Input: part model. Units: mm. Frame: model coordinates. A direction names the side the tool comes from. Give positions to 0.01 mm unless a question says otherwise; leave off trailing zeros. Loops run counter-clockwise (first coordinate to the right, second up) from the corner with the lowest first, then second, coordinate; pieces in that order, holes last.
from build123d import *

# Parameters (mm, degrees)
BASE_PLATE_DEPTH       = 1
UPRIGHT_PLATE_SKETCH_R = 1
UPRIGHT_PLATE_DEPTH    = 1
RIB_SKETCH_W           = 1
RIB_SKETCH_H           = 4
RIB_DEPTH              = 5
PIVOT_HUB_DEPTH        = 1
PIVOT_HUB_DEPTH_BACK   = 2
PIVOT_HUB_SKETCH_R     = 1.5
HUB_BORE_SKETCH_R      = 0.75
HUB_BORE_DEPTH         = 3
SLOT_CUT_DEPTH         = 3


with BuildPart() as part:
    # Base Plate Sketch → Base Plate (new body)
    with BuildSketch(Plane(origin=(0, 0, 0), x_dir=(1, 0, 0), z_dir=(0, 1, 0))):
        with BuildLine():
            Line((-4, 1.5), (-2.8, 1.5))
            ThreePointArc((-2.8, 1.5), (-2.234314575, 1.265685425), (-2, 0.7))
            Line((-2, 0.7), (-2, 0.3))
            ThreePointArc((-2, 0.3), (-2.234314575, -0.265685425), (-2.8, -0.5))
            Line((-2.8, -0.5), (-4, -0.5))
            Line((-4, -0.5), (-4, -3))
            Line((-4, -3), (4, -3))
            Line((4, -3), (4, -0.5))
            Line((4, -0.5), (2.8, -0.5))
            ThreePointArc((2.8, -0.5), (2.234314575, -0.265685425), (2, 0.3))
            Line((2, 0.3), (2, 0.7))
            ThreePointArc((2, 0.7), (2.234314575, 1.265685425), (2.8, 1.5))
            Line((2.8, 1.5), (4, 1.5))
            ThreePointArc((4, 1.5), (3.560660172, 2.560660172), (2.5, 3))
            Line((2.5, 3), (-2.5, 3))
            ThreePointArc((-2.5, 3), (-3.560660172, 2.560660172), (-4, 1.5))
        make_face()
    extrude(amount=BASE_PLATE_DEPTH)

    # Upright Plate Sketch → Upright Plate (add)
    with BuildSketch(Plane.XY.offset(3)):
        with BuildLine():
            Line((-4, 0), (4, 0))
            Line((4, 0), (4, 3))
            ThreePointArc((4, 3), (3.414213562, 4.414213562), (2, 5))
            Line((2, 5), (-2, 5))
            ThreePointArc((-2, 5), (-3.414213562, 4.414213562), (-4, 3))
            Line((-4, 3), (-4, 0))
        make_face()
        with Locations((-2, 3)):
            Circle(UPRIGHT_PLATE_SKETCH_R, mode=Mode.SUBTRACT)
        with Locations((2, 3)):
            Circle(UPRIGHT_PLATE_SKETCH_R, mode=Mode.SUBTRACT)
    extrude(amount=-UPRIGHT_PLATE_DEPTH)

    # Rib Sketch → Rib (add)
    with BuildSketch(Plane(origin=(0, 0, 2), x_dir=(-1, 0, 0), z_dir=(0, 0, -1))):
        with Locations((0.039501807, 3)):
            Rectangle(RIB_SKETCH_W, RIB_SKETCH_H)
    extrude(amount=RIB_DEPTH)

    # Pivot Hub Sketch → Pivot Hub (add, two sides: drawn at the far end of the back side and taken through both)
    with BuildSketch(Plane(origin=(0.460498193, 0, 0), x_dir=(0, 0, -1), z_dir=(1, 0, 0)).offset(-PIVOT_HUB_DEPTH_BACK)):
        with Locations((1.5, 3.5)):
            Circle(PIVOT_HUB_SKETCH_R)
    extrude(amount=PIVOT_HUB_DEPTH + PIVOT_HUB_DEPTH_BACK)

    # Hub Bore Sketch → Hub Bore (cut)
    with BuildSketch(Plane(origin=(1.460498193, 0, 0), x_dir=(0, 0, -1), z_dir=(1, 0, 0))):
        with Locations((1.5, 3.5)):
            Circle(HUB_BORE_SKETCH_R)
    extrude(amount=-HUB_BORE_DEPTH, mode=Mode.SUBTRACT)

    # Slot Cut Sketch → Slot Cut (cut)
    with BuildSketch(Plane(origin=(0.460498193, 0, 0), x_dir=(0, 0, -1), z_dir=(1, 0, 0))):
        with BuildLine():
            Line((1.5, 5), (3, 5))
            Line((3, 5), (3, 3.5))
            ThreePointArc((3, 3.5), (2.560660172, 4.560660172), (1.5, 5))
        make_face()
    extrude(amount=-SLOT_CUT_DEPTH, mode=Mode.SUBTRACT)


solid = part.part
(1) Pin query (flat end, axial travel): pin 1 Ø1.7 at (y, z) = (3.5, -1.5) entering from -X. Return the tip coordinate at first contact, or that it passes through.
Values follow:
pin 1: stops at x = -1.54
(2) Cut plane C-C (y = 1.9). Return the cut outline in (x, z).
Values follow:
outline: (-4, 2) - (-0.54, 2) - (-0.54, -3) - (0.46, -3) - (0.46, 2) - (4, 2) - (4, 3) - (-4, 3) - close
(3) Cut plane D-D (y = 0.4). Return the cut outline in (x, z).
Values follow:
outline: (-4, -1.5) arc R1.5 ccw to (-2.5, -3) - (2.5, -3) arc R1.5 ccw to (4, -1.5) - (2.8, -1.5) arc R0.8 cw to (2, -0.7) - (2, -0.3) arc R0.8 cw to (2.8, 0.5) - (4, 0.5) - (4, 3) - (-4, 3) - (-4, 0.5) - (-2.8, 0.5) arc R0.8 cw to (-2, -0.3) - (-2, -0.7) arc R0.8 cw to (-2.8, -1.5) - close
(4) Mould query, pull axis X, two halves, no side actions, for faces 1 (the cylindrical face through (1.263, 3.676, 2.507)), 2 (the flat face through (-1.54, 2.85, -2.15)), 3 (the cylindrical face through (3.57, 0.49, -2.55)), 4 (the flat face through (-3.4, 0.5, -1.5)). Classes: +X half, -X half, draft (parallel to the pull), parting line (faces both ways), or undercut.
Values follow:
face 1: undercut
face 2: -X half
face 3: +X half
face 4: draft
(5) Reachability of faces 5 (the flat face through (3, 2, 2)), 6 (the flat face through (-1.5, 1, -0.5)), 7 (the flat face through (1.8, 1, -0.5)) from +Z, -Z, +X, -X, +Y, -Y: full face, straight path, thin tool, end or side. Return the list, or none.
Values follow:
face 5: +X, +Y
face 6: -Z, -X
face 7: -Z, +X
(6) Cut plane A-A (y = 3.65). Return the cut outline in (x, z).
Values follow:
outline: (-3.89, 2) - (-2.76, 2) - (-2.76, 3) - (-3.89, 3) - close; (-1.54, -2.99) - (1.46, -2.99) - (1.46, -2.23) - (-1.54, -2.23) - close; (-1.54, -0.77) - (1.46, -0.77) - (1.46, -0.01) - (0.46, -0.01) - (0.46, 2) - (1.24, 2) - (1.24, 3) - (-1.24, 3) - (-1.24, 2) - (-0.54, 2) - (-0.54, -0.01) - (-1.54, -0.01) - close; (2.76, 2) - (3.89, 2) - (3.89, 3) - (2.76, 3) - close
(7) Ray query, probe 1 along Y at (x, z) = (2, 2.7); probe 2 along X at (y, z) = (2.45, 2.35); probe 3 along Z at (x, y) = (0.75, 3.25). Return the intervals inside material, ascending.
Values follow:
probe 1: y = 0 to 2, 4 to 5
probe 2: x = -4 to -2.84, -1.16 to 1.16, 2.84 to 4
probe 3: z = -2.98 to -2.21, -0.79 to -0.02, 2 to 3
